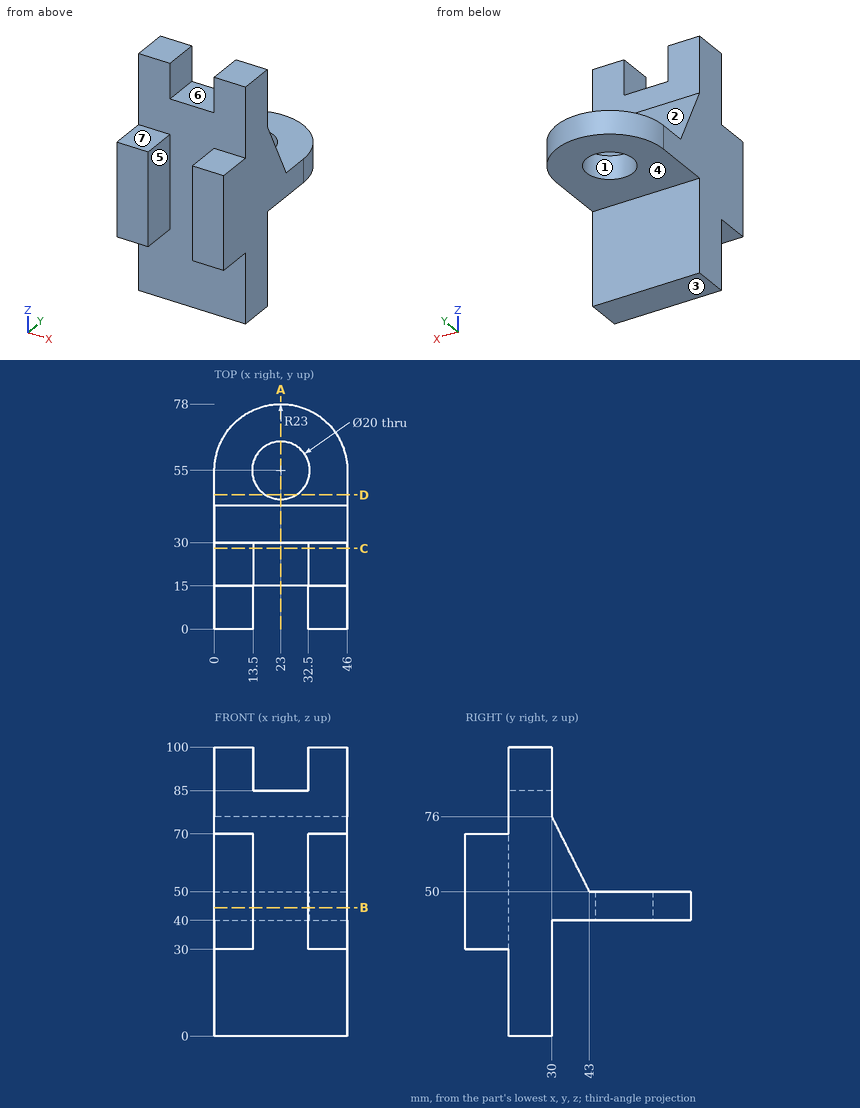
Geometry: see drawing. Coordinates: mm, zero at the bounding-box minimum. A direction names the side the tool comes from. Give positions to 0.01 mm unless a question says otherwise; leave off trailing zeros. Write each loop counter-clockwise with the first axis right and the second up, starting at its lowest first coordinate (ties: lowest second). Pieces come first, ordered by that corner, then holes. Notation, with made-up numbers: (15, -5) -> (22, -5) arc R22 ccw to (22, 22) -> close; hole circle Ø10 at (86.25, 65). An arc over 180 degrees is marked (long way). Use one line per item in the form item = value. Start each with the question number.
1) Ray query, probe 1 along Y at (x, z) = (23, 42); probe 2 along X at (y, z) = (10, 57); probe 3 along Y at (x, z) = (31.5, 33). Return the intervals inside material, ascending. Write a range as from..to.
2) Draft query along Y for the marked faces 1, 2 and 3. Return one class per face: pulls with the +Y half, pulls with the -Y half, needs draft (parallel to the pull), parting line crosses it, or undercut.
3) Section query D-D on y = 46.5. Return the cut outline in (x, z), then the cut area to 3 significant figures.
4) Section query A-A on x = 23. Return the cut outline in (y, z), then the cut area to 3 significant figures.
5) Pin query (flat end, axial travel): pin 1 (11 mm diameter, centred on x = 4.5, y = 7.5, fed in from -Z); pin 2 (16 mm diameter, centred on x = 23, y = 55, fed in from +Z); pin 3 (1.5 mm diameter, centred on x = 25, y = 44, fed in from -Z); pin 4 (15 mm diameter, centred on x = 40.5, y = 7, fed in from +Z). Return the tip coordinate at first contact, or that it passes through.
6) Set-up query: the marked faces 4, 5, 6 and 7. Return all of +Z, -Z, +X, -X, +Y, -Y with unobstructed straight access to the full face (end or side cutting, diameter ignored); none if empty.
7) Section query B-B on z = 44.5. Return the cut outline in (x, y).
8) Section query C-C on y = 28. Return the cut outline in (x, z).
Outcome:
q1.probe_1 = 15..45, 65..78
q1.probe_2 = 0..13.5, 32.5..46
q1.probe_3 = 15..30
q2.face_1 = undercut
q2.face_2 = pulls with the +Y half
q2.face_3 = needs draft
q3.outline = (0, 40) -> (17.73, 40) -> (17.73, 50) -> (0, 50) -> close; (28.27, 40) -> (46, 40) -> (46, 50) -> (28.27, 50) -> close
q3.area = 355 mm^2
q4.outline = (15, 0) -> (30, 0) -> (30, 40) -> (45, 40) -> (45, 50) -> (43, 50) -> (30, 76) -> (30, 85) -> (15, 85) -> close; (65, 40) -> (78, 40) -> (78, 50) -> (65, 50) -> close
q4.area = 1,720 mm^2
q5.pin_1 = 30
q5.pin_2 = through
q5.pin_3 = 40
q5.pin_4 = 70
q6.face_4 = -Z, +X, -X, +Y
q6.face_5 = +Z, -Z, -Y
q6.face_6 = +Z, +Y, -Y
q6.face_7 = +Z, +X, -X, -Y
q7.outline = (0, 0) -> (13.5, 0) -> (13.5, 15) -> (32.5, 15) -> (32.5, 0) -> (46, 0) -> (46, 55) arc R23 ccw to (0, 55) -> close; hole circle Ø20 at (23, 55)
q8.outline = (0, 0) -> (46, 0) -> (46, 100) -> (32.5, 100) -> (32.5, 85) -> (13.5, 85) -> (13.5, 100) -> (0, 100) -> close
